Source: CAD feature listing. Evaluate the final solid. Frame: model axes, mm. A direction names the side the tool comes from. Give positions to 0.01 mm unless a question says otherwise; leave off trailing zeros. Write each loop counter-clockwise with the first axis right and the second up, starting at its lowest first coordinate (ties: lowest second). Pieces come first, ordered by that corner, then holes. Notation, with made-up numbers: (-14.75, 25.5) -> (6.25, 25.5) arc R32 ccw to (6.25, 61.5) -> close; hole circle Ø5 at (65, 3). An arc over 180 degrees is marked (long way). Use one line per item in the form item = value. Start each with the question number.
(1) Cut plane B-B, the plane y = 106. Output: boundary loops of the cut face in (x, z), and give its area (3 significant figures).
(2) Material intervals for line 1 along Y through (x, z) = (38, 10); line 2 along X through (y, z) = (66, 20); line 3 along X through (y, z) = (10.5, 24.5), sorted ascending. Write a range as from..to.
(3) Cut plane C-C, the plane z = 8. Output: boundary loops of the cut face in (x, y), and give its area (3 significant figures).
(4) Draft query along X for faces 6 (the face through (38, 20, 20)), 7 (the face through (-6, 66, 35)), 8 (the face through (38, 119, 10)), 9 (the face through (37.6, 80.7, 30)). Return one class per face: pulls with the +X half, pulls with the -X half, needs draft (parallel to the pull), parting line crosses it, or undercut.
(5) First-contact query: P1, Ø3, axis at x = 95.5, y = 71, coming from the -Z side; P2, Ø3, axis at y = 22, z = 7.5, coming from the -X side; P3, Ø5, axis at x = 64, z = 4.5, coming from the +Y side. Flat tips, straight axial feed; report the tip coordinate or a pass-through.
(6) Cut plane A-A, the plane x = 38. Output: boundary loops of the cut face in (y, z), and give its area (3 significant figures).
(7) Cut plane D-D, the plane y = 86.5. Output: boundary loops of the cut face in (x, z), and give its area (3 significant figures).
(8) Set-up query: faces 1 (the face through (82, 67, 5)), 2 (the face through (-6, 66, 5)), 3 (the face through (0, 32, 20)), 4 (the face through (82, 67, 35)), 5 (the face through (20, 10, 20)). Return all of +Z, -Z, +X, -X, +Y, -Y with unobstructed straight access to the full face (end or side cutting, diameter ignored); none if empty.
from build123d import *

# Parameters (mm, degrees)
BASE_BODY_DEPTH             = 40
UPPER_BODY_DEPTH            = 40
LEFT_LUG_BLOCK_SKETCH_W     = 20
LEFT_LUG_BLOCK_SKETCH_H     = 5
LEFT_LUG_BLOCK_DEPTH        = 19
LEFT_LUG_ARM_SKETCH_W       = 20
LEFT_LUG_ARM_SKETCH_H       = 5
LEFT_LUG_ARM_DEPTH          = 21
LEFT_LUG_ROUNDED_END_DEPTH  = 10
LEFT_LUG_HOLE_SKETCH_R      = 5
LEFT_LUG_HOLE_10_DEPTH      = 10
RIGHT_LUG_BLOCK_SKETCH_W    = 20
RIGHT_LUG_BLOCK_SKETCH_H    = 5
RIGHT_LUG_BLOCK_DEPTH       = 19
RIGHT_LUG_ARM_SKETCH_W      = 20
RIGHT_LUG_ARM_SKETCH_H      = 5
RIGHT_LUG_ARM_DEPTH         = 21
RIGHT_LUG_ROUNDED_END_DEPTH = 10
RIGHT_LUG_HOLE_SKETCH_R     = 5
RIGHT_LUG_HOLE_10_DEPTH     = 10
BEARING_SEAT_CUT_54_DEPTH   = 10
SEAT_GROOVE_38_DEPTH        = 30
HUB_SKETCH_R                = 19
HUB_38_DEPTH                = 30
HUB_RECESS_SKETCH_R         = 19
HUB_RECESS_38_DEPTH         = 10
BORE_SKETCH_R               = 10
BORE_20_DEPTH               = 20


with BuildPart() as part:
    # Base Body Sketch → Base Body (new body)
    with BuildSketch(Plane.XY):
        Polygon((0, 0), (0, 64), (76, 64), (76, 0), (56, 0), (56, 20), (20, 20), (20, 0), align=None)
    extrude(amount=BASE_BODY_DEPTH)

    # Upper Body Sketch → Upper Body (add)
    with BuildSketch(Plane.XY.offset(40)):
        Polygon((0, 64), (-6, 64), (-6, 69), (8, 100), (38, 100), (68, 100), (82, 69), (82, 64), (76, 64), align=None)
    extrude(amount=-UPPER_BODY_DEPTH)

    # Left Lug Block Sketch → Left Lug Block (add)
    with BuildSketch(Plane.ZY.offset(6)):
        with Locations((20, 66.5)):
            Rectangle(LEFT_LUG_BLOCK_SKETCH_W, LEFT_LUG_BLOCK_SKETCH_H)
    extrude(amount=LEFT_LUG_BLOCK_DEPTH)

    # Left Lug Arm Sketch → Left Lug Arm (add)
    with BuildSketch(Plane.ZY.offset(25)):
        with Locations((20, 71.5)):
            Rectangle(LEFT_LUG_ARM_SKETCH_W, LEFT_LUG_ARM_SKETCH_H)
    extrude(amount=-LEFT_LUG_ARM_DEPTH)

    # Left Lug End Sketch → Left Lug Rounded End (add)
    with BuildSketch(Plane(origin=(0, 74, 0), x_dir=(1, 0, 0), z_dir=(0, 1, 0))):
        with BuildLine():
            Line((-25, -10), (-25, -30))
            ThreePointArc((-25, -30), (-35, -20), (-25, -10))
        make_face()
    extrude(amount=-LEFT_LUG_ROUNDED_END_DEPTH)

    # Left Lug Hole Sketch → Left Lug Hole Ø10 (cut)
    with BuildSketch(Plane(origin=(0, 74, 0), x_dir=(1, 0, 0), z_dir=(0, 1, 0))):
        with Locations(Location((-25, -20, 0), (0, 0, 270))):
            Circle(LEFT_LUG_HOLE_SKETCH_R)
    extrude(amount=-LEFT_LUG_HOLE_10_DEPTH, mode=Mode.SUBTRACT)

    # Right Lug Block Sketch → Right Lug Block (add)
    with BuildSketch(Plane(origin=(82, 0, 0), x_dir=(0, 0, -1), z_dir=(1, 0, 0))):
        with Locations((-20, 66.5)):
            Rectangle(RIGHT_LUG_BLOCK_SKETCH_W, RIGHT_LUG_BLOCK_SKETCH_H)
    extrude(amount=RIGHT_LUG_BLOCK_DEPTH)

    # Right Lug Arm Sketch → Right Lug Arm (add)
    with BuildSketch(Plane(origin=(101, 0, 0), x_dir=(0, 0, -1), z_dir=(1, 0, 0))):
        with Locations((-20, 71.5)):
            Rectangle(RIGHT_LUG_ARM_SKETCH_W, RIGHT_LUG_ARM_SKETCH_H)
    extrude(amount=-RIGHT_LUG_ARM_DEPTH)

    # Right Lug End Sketch → Right Lug Rounded End (add)
    with BuildSketch(Plane(origin=(0, 74, 0), x_dir=(1, 0, 0), z_dir=(0, 1, 0))):
        with BuildLine():
            Line((101, -10), (101, -30))
            ThreePointArc((101, -30), (111, -20), (101, -10))
        make_face()
    extrude(amount=-RIGHT_LUG_ROUNDED_END_DEPTH)

    # Right Lug Hole Sketch → Right Lug Hole Ø10 (cut)
    with BuildSketch(Plane(origin=(0, 74, 0), x_dir=(1, 0, 0), z_dir=(0, 1, 0))):
        with Locations(Location((101, -20, 0), (0, 0, 270))):
            Circle(RIGHT_LUG_HOLE_SKETCH_R)
    extrude(amount=-RIGHT_LUG_HOLE_10_DEPTH, mode=Mode.SUBTRACT)

    # Bearing Seat Sketch → Bearing Seat Cut Ø54 (cut)
    with BuildSketch(Plane.XY.offset(40)):
        with BuildLine():
            Line((11, 100), (65, 100))
            ThreePointArc((65, 100), (38, 73), (11, 100))
        make_face()
    extrude(amount=-BEARING_SEAT_CUT_54_DEPTH, mode=Mode.SUBTRACT)

    # Seat Groove Sketch → Seat Groove Ø38 (cut)
    with BuildSketch(Plane.XY.offset(30)):
        with BuildLine():
            Line((19, 100), (57, 100))
            ThreePointArc((57, 100), (38, 81), (19, 100))
        make_face()
    extrude(amount=-SEAT_GROOVE_38_DEPTH, mode=Mode.SUBTRACT)

    # Hub Sketch → Hub Ø38 (add)
    with BuildSketch(Plane.XY.offset(30)):
        with Locations((38, 100)):
            Circle(HUB_SKETCH_R)
    extrude(amount=-HUB_38_DEPTH)

    # Hub Recess Sketch → Hub Recess Ø38 (cut)
    with BuildSketch(Plane.XY.offset(30)):
        with Locations((38, 100)):
            Circle(HUB_RECESS_SKETCH_R)
    extrude(amount=-HUB_RECESS_38_DEPTH, mode=Mode.SUBTRACT)

    # Bore Sketch → Bore Ø20 (cut)
    with BuildSketch(Plane.XY.offset(20)):
        with Locations((38, 100)):
            Circle(BORE_SKETCH_R)
    extrude(amount=-BORE_20_DEPTH, mode=Mode.SUBTRACT)


solid = part.part
Geometry says:
q1.outline = (19.97, 0) -> (30, 0) -> (30, 20) -> (19.97, 20) -> close; (46, 0) -> (56.03, 0) -> (56.03, 20) -> (46, 20) -> close
q1.area = 401 mm^2
q2.line_1 = 20..90, 110..119
q2.line_2 = -35..-30, -20..96, 106..111
q2.line_3 = 0..20, 56..76
q3.outline = (-6, 64) -> (0, 64) -> (0, 0) -> (20, 0) -> (20, 20) -> (56, 20) -> (56, 0) -> (76, 0) -> (76, 64) -> (82, 64) -> (82, 69) -> (68, 100) -> (57, 100) arc R19 ccw to (19, 100) -> (8, 100) -> (-6, 69) -> close; hole circle Ø20 at (38, 100)
q3.area = 7,130 mm^2
q4.face_6 = undercut
q4.face_7 = pulls with the -X half
q4.face_8 = parting line crosses it
q4.face_9 = undercut
q5.P1 = 10
q5.P2 = 0
q5.P3 = 100
q6.outline = (20, 0) -> (90, 0) -> (90, 20) -> (81, 20) -> (81, 30) -> (73, 30) -> (73, 40) -> (20, 40) -> close; (110, 0) -> (119, 0) -> (119, 20) -> (110, 20) -> close
q6.area = 2,720 mm^2
q7.outline = (1.9, 0) -> (74.1, 0) -> (74.1, 40) -> (61.38, 40) -> (61.38, 30) -> (51.37, 30) -> (51.37, 20) -> (24.63, 20) -> (24.63, 30) -> (14.62, 30) -> (14.62, 40) -> (1.9, 40) -> close
q7.area = 2,150 mm^2
q8.face_1 = -Z, +X, +Y, -Y
q8.face_2 = -Z, -X, +Y, -Y
q8.face_3 = +Z, -Z, -X, -Y
q8.face_4 = +Z, +X, +Y, -Y
q8.face_5 = +Z, -Z, -Y
